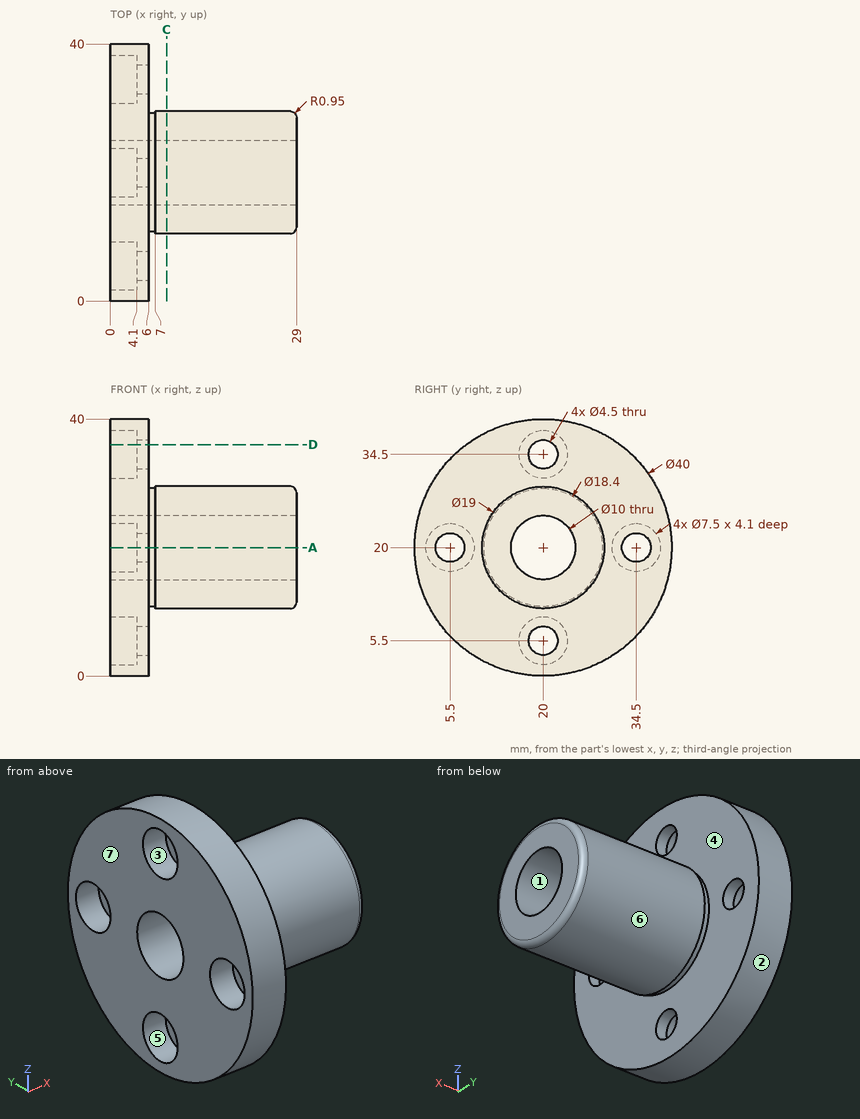
The figure shows three views and two pictorial views of one solid part (mm, origin at its lowest corner). Answer the questions. A direction names the side the tool comes from. Coordinates: 2 decimals unless noted, no trailing zeros. Loops run counter-clockwise (first coordinate to the right, second up) from the corner with the lowest first, then second, coordinate; pieces in that order, holes last. Notation, with made-up numbers: M 49.25,-3 L 82.25,-3 A21 ccw 82.25,27 Z; hole C -34.5,42.25 d2. An arc over 180 degrees is marked long. Answer as CSV lines item,"result". Start each with the question number.
(1) The mould has two halves that part along Z. Classify the marked faces 1, 2, 3 and 4: pulls with the +Z half, pulls with the -Z half, needs draft (parallel to the pull), parting line crosses it, or undercut.
(2) Find the intervals of material crossed by L1, parallel to Y at x = 3, z = 20; L2, parallel to Y at x = 22, z = 20; L3, parallel to X at y = 27.5, z = 35.5, in increasing order. Write a range as [from, to].
(3) Given pin 1 (2 mm diameter, centred on y = 19, z = 35, fed in from -X); pin 2 (6 mm diameter, centred on y = 20, z = 34.5, fed in from +X); pin 3 (4 mm diameter, centred on x = 10.5, z = 22, fed in from -Y); pin 4 (6 mm diameter, centred on y = 20, z = 34.5, fed in from -X), each flat-ended and moving along its own axis, determine where each tip first touches the part or whether it passes through.
(4) The part is cut by section C-C (x = 8.75). Give the vertices of the cut face in (y, z).
(5) The part is cut by section A-A (z = 20). State how many separate pieces and enclosed holes the cut face has, and give its area (3 significant figures).
(6) The part is cut by section D-D (z = 36). Give the vertices of the cut face in (x, y).
(7) For the marked faces 5, 6 and 7, determine the directions among +Z, -Z, +X, -X, +Y, -Y from which every point of the face is accessible in a straight line to the end or side of a thin tool.
Determined:
1,face 1,"undercut"
1,face 2,"parting line crosses it"
1,face 3,"undercut"
1,face 4,"needs draft"
2,L1,"[0, 1.75], [9.25, 15], [25, 30.75], [38.25, 40]"
2,L2,"[10.5, 15], [25, 29.5]"
2,L3,"[0, 6]"
3,pin 1,"through"
3,pin 2,"x = 6"
3,pin 3,"y = 10.5"
3,pin 4,"x = 4.1"
4,outline,"C 20,20 d19; hole C 20,20 d10"
5,separate pieces,"4"
5,enclosed holes,"0"
5,area,"307 mm2"
6,outline,"M 0,8 L 6,8 L 6,18.32 L 4.1,18.32 L 4.1,16.56 L 0,16.56 Z; M 0,23.44 L 4.1,23.44 L 4.1,21.68 L 6,21.68 L 6,32 L 0,32 Z"
7,face 5,"-X"
7,face 6,"+X"
7,face 7,"+Z, -Z, -X, +Y, -Y"
